CAD build for the part. Positions are in the model's coordinates, mm. Face numbers are marked on the shaded views. Round coordinates to 2 decimals unless told otherwise and drop trailing zeros. Loops run counter-clockwise (first coordinate to the right, second up) from the corner with the lowest first, then second, coordinate; pieces in that order, holes last.
from build123d import *

# Parameters (mm, degrees)
SKETCH1_W           = 110
SKETCH1_H           = 110
BOSS_EXTRUDE1_DEPTH = 72
SKETCH2_W           = 40
SKETCH2_H           = 20
CUT_EXTRUDE1_DEPTH  = 10


with BuildPart() as part:
    # Sketch1 → Boss-Extrude1 (new body)
    with BuildSketch(Plane(origin=(0, 0, 0), x_dir=(1, 0, 0), z_dir=(0, 1, 0))):
        Rectangle(SKETCH1_W, SKETCH1_H)
    extrude(amount=BOSS_EXTRUDE1_DEPTH)

    # Sketch2 → Cut-Extrude1 (cut)
    with BuildSketch(Plane.XY.offset(55)):
        with Locations((0, 10)):
            Rectangle(SKETCH2_W, SKETCH2_H)
    extrude(amount=-CUT_EXTRUDE1_DEPTH, mode=Mode.SUBTRACT)


solid = part.part
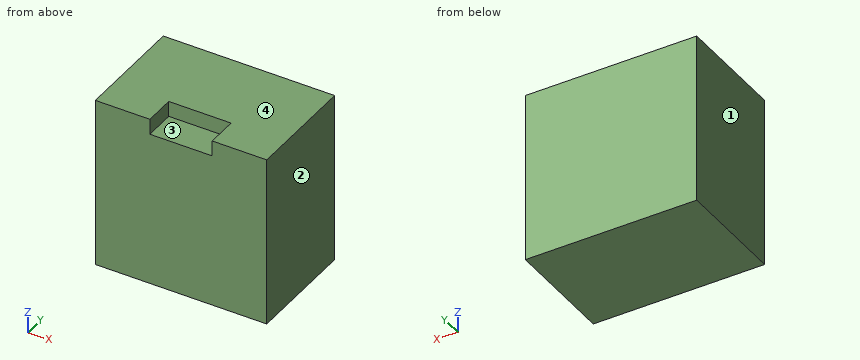
Item 1: Flat gauge pins, fed straight in: P1, Ø3, axis at x = 7, z = 48.5, coming from the -Y side; P2, Ø10, axis at x = -0.5, y = 14.5, coming from the +Z side. Where does each tip first touch, or does it go through?
Verdict:
P1: stops at y = 20
P2: stops at z = 45
Item 2: Wall check: L1, parallel to Z at x = 8, y = 11. Give the ranges that are in metal, low to high.
Verdict:
L1: z = -55 to 45
Item 3: Cut at A-A (x = -17.5). List the corners of the cut face in (y, z).
Verdict:
outline: (0, -55) - (72, -55) - (72, 55) - (20, 55) - (20, 45) - (0, 45) - close
Item 4: Mould opens along X. For the marked faces 1, 2, 3 and 4 say: released by +X, released by -X, zero draft, split by the parting line, or undercut.
Verdict:
face 1: released by -X
face 2: released by +X
face 3: undercut
face 4: zero draft
